Could you check a few things on this model? Use its own coordinates, in mm. Face numbers are marked on the shaded views. A direction names the side the tool comes from. Coordinates: 2 decimals unless noted, no trailing zeros. Order: outer loops, then holes, each group sorted by start corner. A loop starts at its lowest first (then second) coordinate and runs counter-clockwise, first axis right, second up. Notation, with made-up numbers: (23.5, 0.25) - (61.5, 0.25) arc R23 ccw to (61.5, 36.25) - close; hole circle Ø6 at (-30.75, -12). An arc over 180 degrees is marked (long way). One line per item, written item: value. Start each with the question number.
from build123d import *

# Parameters (mm, degrees)
SKETCH1_R             = 11
SKETCH1_R_2           = 5
BOSS_EXTRUDE1_DEPTH   = 3.5
SKETCH1_2_R           = 5
BOSS_EXTRUDE2_DEPTH   = 1.25
SKETCH1_3_R           = 5
BOSS_EXTRUDE3_DEPTH   = 13.5
M8X1_0_TAPPED_HOLE1_D = 7


with BuildPart() as part:
    # Sketch1 → Boss-Extrude1 (new body)
    with BuildSketch(Plane(origin=(0, 0, 0), x_dir=(1, 0, 0), z_dir=(0, 1, 0))):
        with Locations(Location((0, 0, 0), (0, 0, 270))):
            Circle(SKETCH1_R)
        with Locations(Location((0, 0, 0), (0, 0, 270))):
            Circle(SKETCH1_R_2, mode=Mode.SUBTRACT)
    extrude(amount=BOSS_EXTRUDE1_DEPTH)



with BuildPart() as body_2:
    # Sketch1<2> → Boss-Extrude2 (new body)
    with BuildSketch(Plane(origin=(0, 0, 0), x_dir=(1, 0, 0), z_dir=(0, 1, 0))):
        with Locations(Location((0, 0, 0), (0, 0, 270))):
            Circle(SKETCH1_2_R)
    extrude(amount=-BOSS_EXTRUDE2_DEPTH)


with BuildPart() as part_1:
    add(part.part)

    add(body_2.part)  # Boss-Extrude3 merges body 2
    # Sketch1<3> → Boss-Extrude3 (add)
    with BuildSketch(Plane(origin=(0, 0, 0), x_dir=(1, 0, 0), z_dir=(0, 1, 0))):
        with Locations(Location((0, 0, 0), (0, 0, 270))):
            Circle(SKETCH1_3_R)
    extrude(amount=BOSS_EXTRUDE3_DEPTH)

    # M8x1.0 Tapped Hole1 (through all)
    with Locations(Plane.ZX.offset(13.5)):
        with Locations((0, 0)):
            Hole(M8X1_0_TAPPED_HOLE1_D / 2)


solid = part_1.part
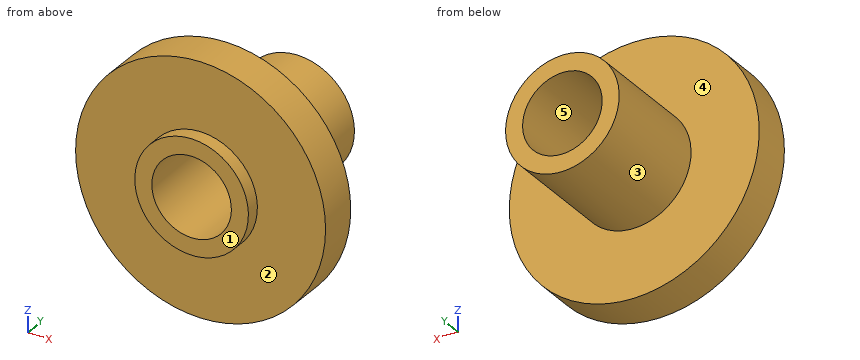
Q1. I want a section at B-B on x = 0. Please give me the cut outline in (y, z), then the cut area to 4 significant figures.
Q2. Which directions (+Z, -Z, +X, -X, +Y, -Y) give clear straight access to the entire face, cutting with the end or side of a thin tool? Please do the marked faces 1 and 2.
Q3. I want a section at C-C on y = 6.75. Please give me the cut outline in (x, z), then the cut area to 3 significant figures.
Q4. I want a section at A-A on z = 0. Please give me the cut outline in (x, y), then the cut area to 4 significant figures.
Q5. If I drill on L1, parallel to X at y = 9.25, z = 0; L2, parallel to X at y = 3, z = 0; L3, parallel to Y at x = -7, z = 2.25, over which ranges is the centre line in solid material (lowest first)?
Q6. We'd pull the mould along Z, two halves only. Please class the marked faces 3, 4 and 5: +Z half, -Z half, draft (parallel to the pull), parting line (faces both ways), or undercut.
Q7. I'm going to push flat-ended pins straight in: pin 1 (4 mm diameter, centred on y = 10, z = -5.5, fed in from -X); pin 2 (3 mm diameter, centred on x = 1.5, y = 5.5, fed in from +Z); pin 3 (3 mm diameter, centred on y = 0.5, z = -2, fed in from -X). Where does each tip first touch, or does it pass through?
Q8. I want a section at D-D on x = 5.75. Please give me the cut outline in (y, z).
Values follow:
1. outline: (-1.25, -5) - (0, -5) - (0, -11) - (3.5, -11) - (3.5, -5) - (13.5, -5) - (13.5, -3.5) - (-1.25, -3.5) - close; (-1.25, 3.5) - (13.5, 3.5) - (13.5, 5) - (3.5, 5) - (3.5, 11) - (0, 11) - (0, 5) - (-1.25, 5) - close
1. area: 86.25 mm^2
2. face 1: +Z, -Z, +X, -X, -Y
2. face 2: -Y
3. outline: circle Ø10 at (0, 0); hole circle Ø7 at (0, 0)
3. area: 40.1 mm^2
4. outline: (-11, 0) - (-5, 0) - (-5, -1.25) - (-3.5, -1.25) - (-3.5, 13.5) - (-5, 13.5) - (-5, 3.5) - (-11, 3.5) - close; (3.5, -1.25) - (5, -1.25) - (5, 0) - (11, 0) - (11, 3.5) - (5, 3.5) - (5, 13.5) - (3.5, 13.5) - close
4. area: 86.25 mm^2
5. L1: x = -5 to -3.5, 3.5 to 5
5. L2: x = -11 to -3.5, 3.5 to 11
5. L3: y = 0 to 3.5
6. face 3: parting line
6. face 4: draft
6. face 5: undercut
7. pin 1: stops at x = -3.57
7. pin 2: stops at z = 5
7. pin 3: stops at x = -10.99
8. outline: (0, -9.38) - (3.5, -9.38) - (3.5, 9.38) - (0, 9.38) - close
